Part model, mm, in its own coordinate system. Face numbers are marked on the shaded views. A direction names the side the tool comes from. Give positions to 0.01 mm unless a question says otherwise; leave off trailing zeros. Write each loop counter-clockwise with the first axis right and the second up, starting at its lowest first coordinate (ties: lowest second). Pieces come first, ordered by that corner, then holes. Notation, with made-up numbers: M 63.5,-16 L 115.5,-16 A24 cw 115.5,17 Z; hole C -30,-36.75 d10. An arc over 180 degrees is marked long. Answer as CSV lines item,"result". Start each with the question number.
Item 1: 3-axis set-ups, long thin cutter, end or side, ignore diameter. For the marked faces 1 and 2: which of +Z, -Z, +X, -X, +Y, -Y reach the whole face in a straight line?
Item 2: Wall check: L1, parallel to X at y = -0.5, z = 5.75; L2, parallel to Y at x = 54.5, z = 3; L3, parallel to Z at x = 63, y = 0.25. Give the ranges that are in metal, low to high. Write a range as from..to.
Item 3: Band-saw the part on A-A, the plane x = 50. List the corners of the cut face in (y, z), then the cut area to 3 significant figures.
Item 4: Pin check, flat tips, straight feed: pin 1 (8 mm diameter, centred on x = 40, z = -1.5, fed in from +Y); pin 2 (6 mm diameter, centred on x = 69, y = -1.5, fed in from +Z); pin 3 (2 mm diameter, centred on x = 28.5, z = -1.5, fed in from -Y). Stop position of each tip, or through.
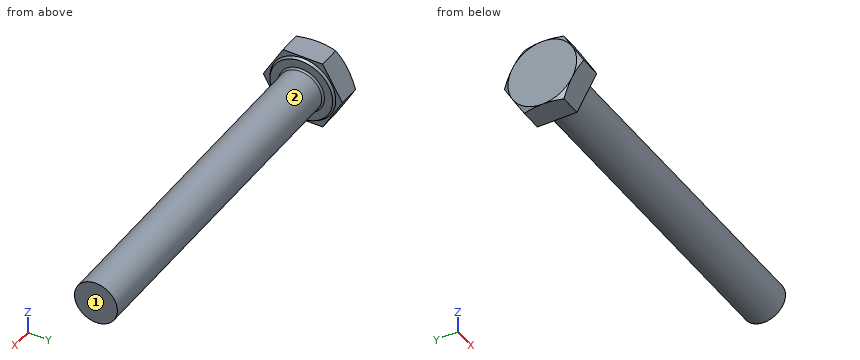
from build123d import *

# Parameters (mm, degrees)
EXTRUDE_384_DEPTH = 6.4
FILLET_1305_R     = 0.4


with BuildPart() as part:
    # 草图1 → Extrude 384 (new body)
    with BuildSketch(Plane(origin=(0, 0, 0), x_dir=(0, 0, -1), z_dir=(1, 0, 0))):
        Polygon((8, 4.618802154), (8, -4.618802154), (0, -9.237604307), (-8, -4.618802154), (-8, 4.618802154), (0, 9.237604307), align=None)
    extrude(amount=EXTRUDE_384_DEPTH)

    # 草图2 → 凸台-旋转1 (revolve)
    with BuildSketch(Plane.XY, mode=Mode.PRIVATE) as revolve_1_sk:
        Polygon((0, 0), (86.4, 0), (86.4, 3.701), (86.4, 5), (60.4, 5), (0, 5), align=None)
    revolve(revolve_1_sk.sketch.rotate(Axis((0, 0, 0), (1, 0, 0)), 90), axis=Axis((0, 0, 0), (1, 0, 0)))

    # 草图3 → 切除-旋转1 (revolve, cut)
    with BuildSketch(Plane.XY):
        Polygon((0, 8), (3.601282526, 14.237604307), (3.601282526, 19.237604307), (-10, 19.237604307), (-10, 8), align=None)
    revolve(axis=Axis((0, 0, 0), (1, 0, 0)), mode=Mode.SUBTRACT)

    # 草图4 → 切除-旋转3 (revolve, cut)
    with BuildSketch(Plane.XY, mode=Mode.PRIVATE) as cut_revolve_3_sk:
        Polygon((6.4, 7.315), (5.8, 7.661410162), (5.8, 9.237604307), (6.4, 9.237604307), align=None)
    revolve(cut_revolve_3_sk.sketch.rotate(Axis((0, 0, 0), (1, 0, 0)), 90), axis=Axis((0, 0, 0), (1, 0, 0)), mode=Mode.SUBTRACT)

    # Fillet 1305
    fillet_1305_edges = [part.edges().sort_by_distance(p)[0] for p in [
        (6.4, 0, -5),
    ]]
    fillet(fillet_1305_edges, radius=FILLET_1305_R)


solid = part.part
Output:
1,face 1,"+Z, -Z, +X, +Y, -Y"
1,face 2,"+X"
2,L1,"0..6.4"
2,L2,"-4..4"
2,L3,"-4.99..4.99"
3,outline,"C 0,0 d10"
3,area,"78.5 mm²"
4,pin 1,"y = 5"
4,pin 2,"z = 5"
4,pin 3,"y = -4.97"
